Here's how the part is built. I have some questions about the finished solid (model axes, mm). A direction names the side the tool comes from. Coordinates: 2 decimals unless noted, no trailing zeros. Loops run counter-clockwise (first coordinate to the right, second up) from the corner with the lowest first, then second, coordinate; pieces in that order, holes last. Notation, with made-up numbers: M 63.5,83 L 93.5,83 A22 cw 93.5,109 Z; hole C -23.5,64 d9. An arc over 180 degrees is marked long. Use one line per item in the form item = value. Start each with the question number.
(1) On a 3-axis mill with a long thin cutter (end or side, diameter ignored), from which of +Z, -Z, +X, -X, +Y, -Y can I reach the whole of each face in a straight line? I mean faces 4 (the cylindrical face through (-222.807, -2.862, 58.944)), 5 (the flat face through (-223, -13, 10)). Say none if no direction works.
(2) Imagine slicing it at A-A, the plane z = 38. Please give me the cut outline in (x, y).
(3) Will these pins go through, and if not, where does the flat tip stop? P1, Ø3, axis at x = -224.5, y = -4, coming from the -Z side; P2, Ø1, axis at x = -227, y = 46, coming from the -Z side; P3, Ø5, axis at x = -220.5, z = 76.5, coming from the +Y side.
(4) Imagine slicing it at C-C, the plane z = 77.5. Please give me the cut outline in (x, y), and give its area (3 significant figures).
(5) Thinking about a two-plate mould opening in Y: for faces 1 (the cylindrical face through (-222.807, -33.979, 91.445)), 2 (the flat face through (-215.412, 63, 62)), 3 (the cylindrical face through (-222.807, 127.979, 41.445)), which applies, +Y half, -Y half, draft (parallel to the pull), parting line (faces both ways), or undercut?
(6) Please list where these lines run through material, in increasing order: L1, parallel to Y at x = -219.5, z = 70; L2, parallel to Y at x = -224.75, z = 7; L3, parallel to Z at x = -229, y = 60.
(7) Imagine slicing it at D-D, the plane y = 92. Please give me the cut outline in (x, z), and give its area (3 significant figures).
(8) Imagine slicing it at B-B, the plane x = -222. Please give me the cut outline in (y, z).
```python
from build123d import *

# Parameters (mm, degrees)
BOSS_EXTRUDE1_DEPTH     = 15
CUT_EXTRUDE1_DEPTH      = 196.228071752
CUT_EXTRUDE1_DEPTH_BACK = 196.228071752
SKETCH3_R               = 15


with BuildPart() as part:
    # Sketch2 → Boss-Extrude1 (new body)
    with BuildSketch(Plane.ZY.offset(215.412167325)):
        with BuildLine():
            Line((0, -13), (20, -13))
            ThreePointArc((20, -13), (41.213203436, -4.213203436), (50, 17))
            Line((50, 17), (50, 107))
            ThreePointArc((50, 107), (41.213203436, 128.213203436), (20, 137))
            Line((20, 137), (0, 137))
            Line((0, 137), (0, 167))
            Line((0, 167), (70, 167))
            ThreePointArc((70, 167), (91.213203436, 158.213203436), (100, 137))
            Line((100, 137), (100, -13))
            ThreePointArc((100, -13), (91.213203436, -34.213203436), (70, -43))
            Line((70, -43), (0, -43))
            Line((0, -43), (0, -13))
        make_face()
    extrude(amount=BOSS_EXTRUDE1_DEPTH)

    # Sketch3 → Cut-Extrude1 (cut, two sides: drawn at the far end of the back side and taken through both)
    with BuildSketch(Plane.ZY.offset(230.412167325).offset(-CUT_EXTRUDE1_DEPTH_BACK)):
        with Locations((70, -13)):
            Circle(SKETCH3_R)
        with Locations((70, 137)):
            Circle(SKETCH3_R)
    extrude(amount=CUT_EXTRUDE1_DEPTH + CUT_EXTRUDE1_DEPTH_BACK, mode=Mode.SUBTRACT)


solid = part.part
```
Answer:
q1.face_4 = +X, -X
q1.face_5 = -Z, +X, -X
q2.outline = M -230.41,-43 L -215.41,-43 L -215.41,-7 L -230.41,-7 Z; M -230.41,131 L -215.41,131 L -215.41,167 L -230.41,167 Z
q3.P1 = 39.84
q3.P2 = 50
q3.P3 = 166.73
q4.outline = M -230.41,-42.05 L -215.41,-42.05 L -215.41,-25.99 L -230.41,-25.99 Z; M -230.41,-0.01 L -215.41,-0.01 L -215.41,124.01 L -230.41,124.01 Z; M -230.41,149.99 L -215.41,149.99 L -215.41,166.05 L -230.41,166.05 Z
q4.area = 2,340 mm²
q5.face_1 = -Y half
q5.face_2 = draft
q5.face_3 = undercut
q6.L1 = -43 to -28, 2 to 122, 152 to 167
q6.L2 = -43 to -13, 137 to 167
q6.L3 = 50 to 100
q7.outline = M -230.41,50 L -215.41,50 L -215.41,100 L -230.41,100 Z
q7.area = 750 mm²
q8.outline = M -43,0 L -13,0 L -13,20 A30 cw 17,50 L 107,50 A30 cw 137,20 L 137,0 L 167,0 L 167,70 A30 ccw 137,100 L -13,100 A30 ccw -43,70 Z; hole C -13,70 d30; hole C 137,70 d30
